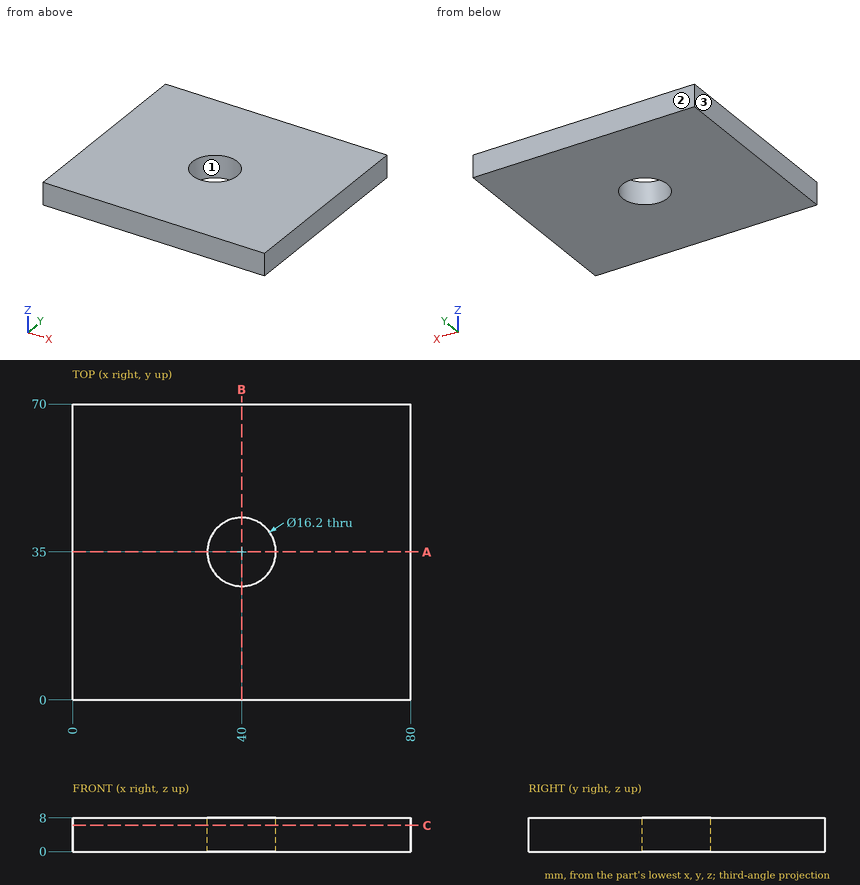
The figure shows three views and two pictorial views of one solid part (mm, origin at its lowest corner). Answer the questions. Round coordinates to 2 decimals unless told otherwise and drop trailing zeros. Write each loop counter-clockwise with the first axis right and the second up, starting at its lowest first coordinate (ties: lowest second). Pieces come first, ordered by that corner, then holes. Notation, with made-up numbers: M 48.5,27.25 L 72.5,27.25 A18 ccw 72.5,58.25 Z; hole C -19,16 d2. An arc over 180 degrees is marked long. Use a Markdown table: item, result.
1) The part is cut by section B-B on x = 40. Give the vertices of the cut face in (y, z).
Taken from the geometry:
| item | result |
|---|---|
| outline | M 0,0 L 26.9,0 L 26.9,8 L 0,8 Z; M 43.1,0 L 70,0 L 70,8 L 43.1,8 Z |
2) Determine the mould class of the marked faces 1, 2 and 3 for opening direction X: pulls with the +X half, pulls with the -X half, needs draft (parallel to the pull), parting line crosses it, or undercut.
Taken from the geometry:
| item | result |
|---|---|
| face 1 | undercut |
| face 2 | needs draft |
| face 3 | pulls with the -X half |
3) The part is cut by section C-C on z = 6.25. Give the vertices of the cut face in (x, y), plus the area to 3 significant figures.
Taken from the geometry:
| item | result |
|---|---|
| outline | M 0,0 L 80,0 L 80,70 L 0,70 Z; hole C 40,35 d16.2 |
| area | 5,390 mm2 |
4) The part is cut by section A-A on y = 35. Give the vertices of the cut face in (x, z), plus the area to 3 significant figures.
Taken from the geometry:
| item | result |
|---|---|
| outline | M 0,0 L 31.9,0 L 31.9,8 L 0,8 Z; M 48.1,0 L 80,0 L 80,8 L 48.1,8 Z |
| area | 510 mm2 |
5) Consider line 1 (Y direction, x = 40, z = 5.5); line 2 (X direction, y = 36.5, z = 1); line 3 (Y direction, x = 33, z = 1). Determine where each line is inside the solid, lowest interval first. Write a range as [from, to].
Taken from the geometry:
| item | result |
|---|---|
| line 1 | y = [0, 26.9], [43.1, 70] |
| line 2 | x = [0, 32.04], [47.96, 80] |
| line 3 | y = [0, 30.92], [39.08, 70] |
